Geometry: final body of the model. Coordinates: model frame, mm. Face numbers are marked on the shaded views. A direction names the side the tool comes from. Coordinates: 2 decimals unless noted, no trailing zeros. Write each loop counter-clockwise with the first axis right and the second up, starting at its lowest first coordinate (ties: lowest second). Pieces come first, ordered by that corner, then holes. Notation, with made-up numbers: (60.5, 81.5) - (103.5, 81.5) arc R37 cw to (103.5, 120.5) - close; hole circle Ø4 at (72, 45). An arc over 180 degrees is marked (long way). Answer as a JSON object with one key per item and string values. Group by question number.
Item 1: First-contact query: pin 1 Ø3 at (x, z) = (-3, 45) entering from +Y; pin 2 Ø6 at (y, z) = (-1.5, 61.5) entering from +X; pin 3 Ø6 at (x, y) = (0, -1) entering from -Z; pin 4 Ø3 at (x, z) = (3.5, 29.5) entering from -Y. Flat tips, straight axial feed; report the tip coordinate or a pass-through.
Item 2: Set-up query: the marked faces 1 and 2. Return all of +Z, -Z, +X, -X, +Y, -Y with unobstructed straight access to the full face (end or side cutting, diameter ignored); none if empty.
Item 3: Line query: line 1 along Z through (x, y) = (5.5, 0.75); line 2 along Y through (x, z) = (3.5, 2); line 3 along Y through (x, z) = (2.5, 15). Output: solid intervals per line, ascending. Write a range as from..to.
Item 4: Section A-A on x = 0. Return loops of the section in (y, z).
Item 5: Section B-B on z = 92.5. Return loops of the section in (x, y), and give its area (3 significant figures).
```python
from build123d import *

# Parameters (mm, degrees)
SKETCH_1_R                = 6.5
EXTRUDE_1_DEPTH           = 20
CHAMFER_1_SIZE            = 0.5
HOLE_WIZARD_2_0_2_1_D     = 2
HOLE_WIZARD_2_0_2_1_DEPTH = 5
HOLE_WIZARD_2_0_2_1_TIP   = 0.600860619
SKETCH_8_R                = 4
EXTRUDE_2_DEPTH           = 105
SKETCH_9_R                = 3
EXTRUDE_3_DEPTH           = 10


with BuildPart() as part:
    # 草图1 → 凸台-拉伸1 (new body)
    with BuildSketch(Plane.XY):
        Circle(SKETCH_1_R)
    extrude(amount=EXTRUDE_1_DEPTH)

    # 倒角1
    chamfer_1_edges = [part.edges().sort_by_distance(p)[0] for p in [
        (-6.5, 0, 0),
    ]]
    chamfer(chamfer_1_edges, length=CHAMFER_1_SIZE)

    # Ø2.0 (2) 直径孔1
    with Locations(Plane(origin=(0, 0, 0), x_dir=(-1, 0, 0), z_dir=(0, 0, -1))):
        with Locations((-3.5, 0), (3.5, 0)):
            Hole(HOLE_WIZARD_2_0_2_1_D / 2, depth=HOLE_WIZARD_2_0_2_1_DEPTH)
            with Locations((0, 0, -(HOLE_WIZARD_2_0_2_1_DEPTH + HOLE_WIZARD_2_0_2_1_TIP / 2))):  # 118° drill point
                Cone(0, HOLE_WIZARD_2_0_2_1_D / 2, HOLE_WIZARD_2_0_2_1_TIP, mode=Mode.SUBTRACT)

    # 草图8 → 凸台-拉伸2 (add)
    with BuildSketch(Plane.XY.offset(20)):
        Circle(SKETCH_8_R)
    extrude(amount=EXTRUDE_2_DEPTH)

    # 草图9 → 凸台-拉伸3 (add)
    with BuildSketch(Plane.XY.offset(125)):
        Circle(SKETCH_9_R)
    extrude(amount=EXTRUDE_3_DEPTH)


solid = part.part
```
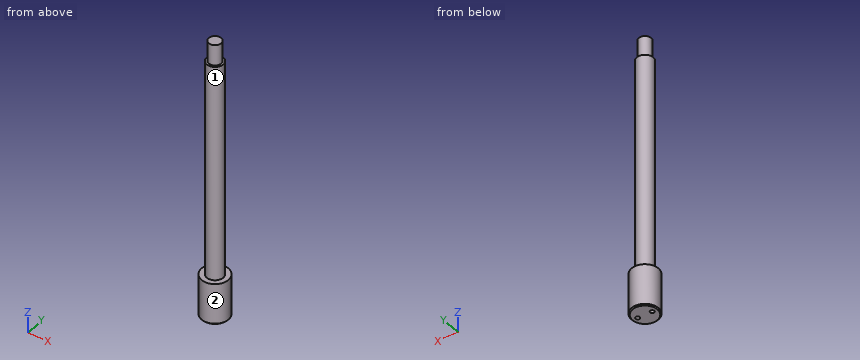
Checks:
{
 "1": {"pin 1": "y = 3.71", "pin 2": "x = 4", "pin 3": "z = 0", "pin 4": "y = -3.46"},
 "2": {"face 1": "+Z", "face 2": "+Z, -Z"},
 "3": {"line 1": "0..20", "line 2": "-5.48..-1, 1..5.48", "line 3": "-6..6"},
 "4": {"outline": "(-6.5, 0.5) - (-6, 0) - (6, 0) - (6.5, 0.5) - (6.5, 20) - (4, 20) - (4, 125) - (3, 125) - (3, 135) - (-3, 135) - (-3, 125) - (-4, 125) - (-4, 20) - (-6.5, 20) - close"},
 "5": {"outline": "circle Ø8 at (0, 0)", "area": "50.3 mm^2"}
}
